The listing builds one solid part. Answer for the finished solid, in the listing's coordinates (mm). A direction names the side the tool comes from. Coordinates: 2 decimals unless noted, no trailing zeros. Order: outer loops, then holes, each group sorted by start corner. A loop starts at its lowest first (then second) coordinate and runs counter-clockwise, first axis right, second up. Notation, with made-up numbers: (88.25, -15) - (124.25, -15) arc R25 ccw to (124.25, 15) - close; hole circle Ø5 at (-28.5, -24.5). An arc over 180 degrees is marked (long way). One line per item, written item: value. Start each with the question number.
```python
from build123d import *
from build123d.topology import SkipClean

# Parameters (mm, degrees)
SKETCH_1_R          = 6
EXTRUDE_1_DEPTH     = 14
SKETCH_2_R          = 7.5
EXTRUDE_2_DEPTH     = 3
SKETCH_3_R          = 5
EXTRUDE_3_DEPTH     = 8
SKETCH_8_R          = 2.1
CUT_EXTRUDE_1_DEPTH = 28.156951228
CHAMFER_1_SIZE      = 0.5
SKETCH_9_W          = 14.77232069
SKETCH_9_H          = 13.551998546
CUT_EXTRUDE_2_DEPTH = 4.5
CHAMFER_2_SIZE      = 0.5
SKETCH_11_W         = 9.643873146
SKETCH_11_H         = 27.541523797
SKETCH_11_W_2       = 13.856983611
CUT_EXTRUDE_3_DEPTH = 10
SKETCH_12_W         = 9.292809808
SKETCH_12_H         = 2
SKETCH_13_W         = 6.810956272
SKETCH_13_H         = 2


with BuildPart() as part:
    # 草图1 → 凸台-拉伸1 (new body)
    with BuildSketch(Plane(origin=(0, 0, 0), x_dir=(1, 0, 0), z_dir=(0, 1, 0))):
        with Locations(Location((0, 0, 0), (0, 0, 270))):
            Circle(SKETCH_1_R)
    extrude(amount=-EXTRUDE_1_DEPTH)

    # 草图2 → 凸台-拉伸2 (add)
    with BuildSketch(Plane.XZ.offset(14)):
        with Locations(Location((0, 0, 0), (0, 0, 270))):
            Circle(SKETCH_2_R)
    extrude(amount=EXTRUDE_2_DEPTH)

    # 草图3 → 凸台-拉伸3 (add)
    with BuildSketch(Plane.XZ.offset(17)):
        with Locations(Location((0, 0, 0), (0, 0, 270))):
            Circle(SKETCH_3_R)
    extrude(amount=EXTRUDE_3_DEPTH)

    # 草图8 → 切除-拉伸1 (cut, through all)
    with BuildSketch(Plane.XZ):
        with Locations(Location((0, 0, 0), (0, 0, 270))):
            Circle(SKETCH_8_R)
    extrude(amount=CUT_EXTRUDE_1_DEPTH, mode=Mode.SUBTRACT)

    # 倒角1
    chamfer_1_edges = [part.edges().sort_by_distance(p)[0] for p in [
        (0, 0, -6),
        (0, -14, 7.5),
        (0, -17, 7.5),
    ]]
    chamfer(chamfer_1_edges, length=CHAMFER_1_SIZE)

    # 草图9 → 切除-拉伸2 (cut, symmetric)
    with SkipClean():  # the faces are left unmerged after this step: merging them gives an invalid solid
        with BuildSketch(Plane.XY):
            with Locations((14.386160345, -10.910714622)):
                Rectangle(SKETCH_9_W, SKETCH_9_H)
        cut_extrude_2 = extrude(amount=CUT_EXTRUDE_2_DEPTH, both=True, mode=Mode.SUBTRACT)

    # 镜向1: 切除-拉伸2 across plane
    add(cut_extrude_2.mirror(Plane(origin=(0, 0, 0), x_dir=(0, 0, 1), z_dir=(1, 0, 0))), mode=Mode.SUBTRACT)

    # 倒角2
    chamfer_2_edges = [part.edges().sort_by_distance(p)[0] for p in [
        (0, -25, 5),
    ]]
    chamfer(chamfer_2_edges, length=CHAMFER_2_SIZE)

    # 草图11 → 切除-拉伸3 (cut, symmetric)
    with BuildSketch(Plane.XY):
        with Locations((10.321936573, -0.229238102)):
            Rectangle(SKETCH_11_W, SKETCH_11_H)
        with Locations((-12.428491806, -0.229238102)):
            Rectangle(SKETCH_11_W_2, SKETCH_11_H)
    extrude(amount=CUT_EXTRUDE_3_DEPTH, both=True, mode=Mode.SUBTRACT)

    # 草图12 → 切除-旋转2 (revolve, cut)
    with BuildSketch(Plane.XY, mode=Mode.PRIVATE) as cut_revolve_2_sk:
        with Locations((-8.646404904, -18)):
            Rectangle(SKETCH_12_W, SKETCH_12_H)
    revolve(cut_revolve_2_sk.sketch.rotate(Axis((0, -17, 0), (0, 1, 0)), 90), axis=Axis((0, -17, 0), (0, 1, 0)), mode=Mode.SUBTRACT)

    # 草图13 → 切除-旋转3 (revolve, cut)
    with BuildSketch(Plane.XY, mode=Mode.PRIVATE) as cut_revolve_3_sk:
        with Locations((-7.905478136, -13)):
            Rectangle(SKETCH_13_W, SKETCH_13_H)
    revolve(cut_revolve_3_sk.sketch.rotate(Axis((0, -14, 0), (0, 1, 0)), 270), axis=Axis((0, -14, 0), (0, 1, 0)), mode=Mode.SUBTRACT)


solid = part.part
```
(1) Flat-ended cylindrical pins translate along their axes: pin 1 Ø3 at (y, z) = (-4, 3) entering from -X; pin 2 Ø2.5 at (y, z) = (-3.5, 1) entering from +X; pin 3 Ø6 at (y, z) = (-19, -5) entering from -X. Find the tip coordinate at first contact, or state that the pin passes through.
(2) For a pull along Y with two mould halves and no side action, classify faces 4 (the face through (-4.88, -21.71, 1.08)), 5 (the face through (0.157, -16.865, 7.134)), 6 (the face through (-5, -14, 0)) as pulls with the +Y half, pulls with the -Y half, needs draft (parallel to the pull), parting line crosses it, or undercut.
(3) The part is cut by section B-B on y = -8.5. Determine the outline of the cut face in (x, z).
(4) For faces 1 (the face through (0, -6, -6)), 2 (the face through (-3, -17, -3)), 3 (the face through (5.5, -6, 0)), determine the directions among +Z, -Z, +X, -X, +Y, -Y from which every point of the face is accessible in a straight line to the end or side of a thin tool.
(5) Consider probe 1 along X at (y, z) = (-5.25, 0); probe 2 along Y at (x, z) = (-4.75, 0.5); probe 3 along Z at (x, y) = (0, -15.25). Determine where each line is inside the solid, lowest interval first.
(6) The part is cut by section C-C on y = -23.5. Determine the outline of the cut face in (x, z).
Completed:
1. pin 1: stops at x = -5.5
1. pin 2: stops at x = 5.5
1. pin 3: stops at x = -6.71
2. face 4: needs draft
2. face 5: pulls with the -Y half
2. face 6: undercut
3. outline: (-5.5, -2.4) arc R6 ccw to (5.5, -2.4) - (5.5, 2.4) arc R6 ccw to (-5.5, 2.4) - close; hole circle Ø4.2 at (0, 0)
4. face 1: -Z, +Y
4. face 2: none
4. face 3: +Z, -Z, +X, +Y
5. probe 1: x = -5.5 to -2.1, 2.1 to 5.5
5. probe 2: y = -24.72 to -19, -17 to -14, -12 to 0
5. probe 3: z = -7.5 to -2.1, 2.1 to 7.5
6. outline: circle Ø10 at (0, 0); hole circle Ø4.2 at (0, 0)
